from build123d import *

# Parameters (mm, degrees)
SKETCH1_R           = 72.5
SKETCH1_R_2         = 4.25
BOSS_EXTRUDE1_DEPTH = 6


with BuildPart() as part:
    # Sketch1 → Boss-Extrude1 (new body)
    with BuildSketch(Plane.XY):
        Circle(SKETCH1_R)
        with Locations((0, 60)):
            Circle(SKETCH1_R_2, mode=Mode.SUBTRACT)
        with Locations((51.961524227, 30)):
            Circle(SKETCH1_R_2, mode=Mode.SUBTRACT)
        with Locations((51.961524227, -30)):
            Circle(SKETCH1_R_2, mode=Mode.SUBTRACT)
        with Locations((0, -60)):
            Circle(SKETCH1_R_2, mode=Mode.SUBTRACT)
        with Locations((-51.961524227, -30)):
            Circle(SKETCH1_R_2, mode=Mode.SUBTRACT)
        with Locations((-51.961524227, 30)):
            Circle(SKETCH1_R_2, mode=Mode.SUBTRACT)
    extrude(amount=BOSS_EXTRUDE1_DEPTH)


solid = part.part
The listing builds one solid part. Answer for the finished solid, in the listing's coordinates (mm). Give positions to 0.01 mm unless a question says otherwise; leave off trailing zeros. Write each loop counter-clockwise with the first axis right and the second up, starting at its lowest first coordinate (ties: lowest second). Pieces come first, ordered by that corner, then holes.
Item 1: Section C-C, the plane z = 1.75 is taken. Write down the section's boundary in (x, y).
Item 2: Find the intervals of material crossed by line 1 along Y through (x, z) = (0, 3.9); line 2 along Y through (x, z) = (-55, 4.25); line 3 along X through (y, z) = (49.5, 2.6), in increasing order.
Item 3: Section B-B, the plane y = -60 is taken. Write down the section's boundary in (x, z), plus the area to 3 significant figures.
Item 4: Section D-D, the plane y = -30 is taken. Write down the section's boundary in (x, z), plus the area to 3 significant figures.
Item 5: Determine the mould class of faces 1 (the cylindrical face through (-50, -33.77, 2.96)), 2 (the cylindrical face through (-50, 26.23, 2.96)), 3 (the cylindrical face through (69.15, 21.78, 2.96)), 4 (the flat face through (-1, 1, 6)) for opening direction Y: released by +Y, released by -Y, zero draft, split by the parting line, or undercut.
Item 6: Section A-A, the plane x = 0 is taken. Write down the section's boundary in (y, z), plus the area to 3 significant figures.
Item 7: Flat-ended cylindrical pins translate along their axes: P1, Ø1, axis at x = -55.5, z = 2, coming from the +Y side; P2, Ø7, axis at x = -51.96, y = -30, coming from the -Z side; P3, Ø1.5, axis at x = 42, z = 4.5, coming from the +Y side. Find the tip coordinate at first contact, or state that the pin passes through.
Completed:
1. outline: circle Ø145 at (0, 0); hole circle Ø8.5 at (-51.96, -30); hole circle Ø8.5 at (-51.96, 30); hole circle Ø8.5 at (0, -60); hole circle Ø8.5 at (0, 60); hole circle Ø8.5 at (51.96, -30); hole circle Ø8.5 at (51.96, 30)
2. line 1: y = -72.5 to -64.25, -55.75 to 55.75, 64.25 to 72.5
2. line 2: y = -47.24 to -32.97, -27.03 to 27.03, 32.97 to 47.24
2. line 3: x = -52.97 to 52.97
3. outline: (-40.7, 0) - (-4.25, 0) - (-4.25, 6) - (-40.7, 6) - close; (4.25, 0) - (40.7, 0) - (40.7, 6) - (4.25, 6) - close
3. area: 437 mm2
4. outline: (-66, 0) - (-56.21, 0) - (-56.21, 6) - (-66, 6) - close; (-47.71, 0) - (47.71, 0) - (47.71, 6) - (-47.71, 6) - close; (56.21, 0) - (66, 0) - (66, 6) - (56.21, 6) - close
4. area: 690 mm2
5. face 1: undercut
5. face 2: undercut
5. face 3: split by the parting line
5. face 4: zero draft
6. outline: (-72.5, 0) - (-64.25, 0) - (-64.25, 6) - (-72.5, 6) - close; (-55.75, 0) - (55.75, 0) - (55.75, 6) - (-55.75, 6) - close; (64.25, 0) - (72.5, 0) - (72.5, 6) - (64.25, 6) - close
6. area: 768 mm2
7. P1: stops at y = 47.24
7. P2: passes through
7. P3: stops at y = 59.62
